Here's how the part is built. I have some questions about the finished solid (model axes, mm). A direction names the side the tool comes from. Give positions to 0.01 mm unless a question says otherwise; leave off trailing zeros. Write each loop counter-clockwise with the first axis right and the second up, starting at its lowest first coordinate (ties: lowest second). Pieces come first, ordered by that corner, then holes. Notation, with made-up numbers: (25.25, 55) - (79.25, 55) arc R34 cw to (79.25, 86) - close; hole circle Ø1 at (-5, 9.25). An arc over 180 degrees is marked (long way). One line per item, written item: value. Start each with the question number.
1) Imagine slicing it at B-B on y = 90. Write out the boundary of the cut face in (x, z).
2) Imagine slicing it at A-A on x = 0. Write out the boundary of the cut face in (y, z).
3) I'm going to push flat-ended pins straight in: P1, Ø12, axis at y = 177, z = 3, coming from the +X side; P2, Ø1, axis at x = 16, z = 12, coming from the +Y side; P3, Ø3, axis at y = 157, z = -12.5, coming from the -X side (3 decimals). Where does each tip first touch, or does it pass through?
4) Please list where these lines run through material, in increasing order: L1, parallel to X at y = 24.5, z = 16; L2, parallel to Y at x = -24, z = -1; L3, parallel to Y at x = -9, z = -2. Write a range as [from, to].
5) On a 3-axis mill with a long thin cutter (end or side, diameter ignored), from which of +Z, -Z, +X, -X, +Y, -Y can I reach the whole of each face in a straight line? I mean faces 4 (the cylindrical face through (0.4, -9.76, 2.17)), 5 (the cylindrical face through (-31.46, 64.18, 4.47)), 6 (the flat face through (0.399, 124.758, 4.504)). Say none if no direction works.
6) Imagine slicing it at D-D on z = 19. Write out the boundary of the cut face in (x, y), plus the area to 3 significant figures.
7) We'd pull the mould along X, two halves only. Please class faces 1 (the flat face through (28.5, 57, 20)), 2 (the cylindrical face through (31.54, 64.18, 4.47)), 3 (the cylindrical face through (-3, 177.93, -9.54)): +X half, -X half, draft (parallel to the pull), parting line (faces both ways), or undercut.
8) Imagine slicing it at C-C on z = 0. Write out the boundary of the cut face in (x, y).
from build123d import *

# Parameters (mm, degrees)
BOSS_EXTRUDE1_DEPTH             = 34.5
SKETCH2_R                       = 100
CUT_EXTRUDE1_DEPTH              = 28.5
CUT_EXTRUDE2_DEPTH              = 57
SKETCH5_R                       = 10
BOSS_EXTRUDE2_DEPTH             = 29
BOSS_EXTRUDE3_REACH             = 229.088
BOSS_EXTRUDE3_END_RADIUS        = 20
SKETCH7_R                       = 10
BOSS_EXTRUDE3_DIRECTION_2_DEPTH = 10


with BuildPart() as part:
    # Sketch1 → Boss-Extrude1 (new, symmetric)
    with BuildSketch(Plane(origin=(0, 0, 0), x_dir=(0, 0, -1), z_dir=(1, 0, 0))):
        with BuildLine():
            ThreePointArc((-16.232839847, 142.89001702), (-44.477266745, 64.681536406), (-15.103918242, -13.10998298))
            ThreePointArc((-15.103918242, -13.10998298), (13.10998298, -15.103918242), (15.103918242, 13.10998298))
            ThreePointArc((15.103918242, 13.10998298), (-4.478314094, 64.970995905), (14.351303838, 117.10998298))
            ThreePointArc((14.351303838, 117.10998298), (11.949249015, 145.292071843), (-16.232839847, 142.89001702))
        make_face()
    extrude(amount=BOSS_EXTRUDE1_DEPTH, both=True)

    # Sketch2 → Cut-Extrude1 (cut, symmetric)
    with BuildSketch(Plane(origin=(0, 0, 0), x_dir=(0, 0, -1), z_dir=(1, 0, 0))):
        Circle(SKETCH2_R)
    extrude(amount=CUT_EXTRUDE1_DEPTH, both=True, mode=Mode.SUBTRACT)

    # Sketch4 → Cut-Extrude2 (cut)
    with BuildSketch(Plane.ZY.offset(-28.5)):
        Polygon((-31.404068156, 111.748185713), (46.911557074, 140.123412246), (75.162269232, 67.90846072), (-19.75286352, 46.910793085), align=None)
    extrude(amount=CUT_EXTRUDE2_DEPTH, mode=Mode.SUBTRACT)

    # Sketch5 → Boss-Extrude2 (add, symmetric)
    with BuildSketch(Plane(origin=(0, 0, 0), x_dir=(0, 0, -1), z_dir=(1, 0, 0))):
        Circle(SKETCH5_R)
    extrude(amount=BOSS_EXTRUDE2_DEPTH, both=True)

    # Boss-Extrude3: up to this cylinder (the profile starts outside it)
    boss_extrude3_end = Plane(origin=(0, 130, 0.940768004), z_dir=(-1, 0, 0)) * Cylinder(BOSS_EXTRUDE3_END_RADIUS, 499.176, mode=Mode.PRIVATE)
    # Sketch7 → Boss-Extrude3 (add, up to the surface)
    with BuildSketch(Plane(origin=(0, 200, 0), x_dir=(1, 0, 0), z_dir=(0, 1, 0)), mode=Mode.PRIVATE) as boss_extrude3_sk1:
        with Locations(Location((0, 0, 0), (0, 0, 90))):
            Circle(SKETCH7_R)
    boss_extrude3_tool1 = extrude(boss_extrude3_sk1.sketch, amount=-BOSS_EXTRUDE3_REACH, mode=Mode.PRIVATE) - boss_extrude3_end
    add(boss_extrude3_tool1.solids().sort_by_distance((0, 200, 0))[0])

    # Sketch7 → Boss-Extrude3 direction 2 (add)
    with BuildSketch(Plane(origin=(0, 200, 0), x_dir=(1, 0, 0), z_dir=(0, 1, 0))):
        with Locations(Location((0, 0, 0), (0, 0, 90))):
            Circle(SKETCH7_R)
    extrude(amount=BOSS_EXTRUDE3_DIRECTION_2_DEPTH)


solid = part.part
Numbers:
1. outline: (-34.5, 0.65) - (-28.5, 0.65) - (-28.5, 41.96) - (-34.5, 41.96) - close; (28.5, 0.65) - (34.5, 0.65) - (34.5, 41.96) - (28.5, 41.96) - close
2. outline: circle Ø20 at (0, 0); (117.74, -14.86) arc R20 ccw to (146.74, -10) - (210, -10) - (210, 10) - (147.83, 10) arc R20 ccw to (142.89, 16.23) arc R120 ccw to (131.97, 24.42) - close
3. P1: x = 10
3. P2: y = 146.99
3. P3: through
4. L1: [-34.5, -28.5], [28.5, 34.5]
4. L2: [-9.95, 9.95], [122.76, 149.91]
4. L3: [-9.8, 9.8], [122.4, 210]
5. face 4: none
5. face 5: -Z, +X, -X
5. face 6: +Z
6. outline: (-34.5, -8.38) - (-28.5, -8.38) - (-28.5, 130.01) - (28.5, 130.01) - (28.5, -8.38) - (34.5, -8.38) - (34.5, 139.48) - (-34.5, 139.48) - close
6. area: 2,310 mm^2
7. face 1: undercut
7. face 2: draft
7. face 3: parting line
8. outline: (-34.5, -20) - (-28.5, -20) - (-28.5, -10) - (28.5, -10) - (28.5, -20) - (34.5, -20) - (34.5, 39.15) - (28.5, 39.15) - (28.5, 10) - (-28.5, 10) - (-28.5, 39.15) - (-34.5, 39.15) - close; (-34.5, 91.95) - (-28.5, 91.95) - (-28.5, 123.13) - (28.5, 123.13) - (28.5, 91.95) - (34.5, 91.95) - (34.5, 149.98) - (10, 149.98) - (10, 210) - (-10, 210) - (-10, 149.98) - (-34.5, 149.98) - close
